Input: part model. Units: mm. Frame: model coordinates. A direction names the side the tool comes from. Round coordinates to 2 decimals unless told otherwise and drop trailing zeros. Write each loop counter-clockwise with the first axis right and the second up, starting at its lowest first coordinate (ties: lowest second). Pieces come first, ordered by that corner, then holes. Notation, with made-up numbers: M 40.5,25 L 78.5,25 A23 cw 78.5,56 Z; hole C 84,8.5 d2. An arc over 180 degrees is marked long. Write each question's results on one line, items separated by ' | '. Start each with the question number.
```python
from build123d import *

# Parameters (mm, degrees)
SKETCH1_W          = 100
SKETCH1_H          = 15
EXTRUDE1_DEPTH     = 15
CUT_EXTRUDE1_DEPTH = 53.737557774
CHAMFER1_SIZE      = 0.5


with BuildPart() as part:
    # Sketch1 → Extrude1 (new body)
    with BuildSketch(Plane(origin=(0, 0, 0), x_dir=(1, 0, 0), z_dir=(0, 1, 0))):
        Rectangle(SKETCH1_W, SKETCH1_H)
    extrude(amount=EXTRUDE1_DEPTH)

    # Sketch4 → Cut-Extrude1 (cut, through all)
    with BuildSketch(Plane(origin=(0, 15, 0), x_dir=(1, 0, 0), z_dir=(0, 1, 0))):
        with BuildLine():
            Line((-42.25, 2.5), (-42.25, -2.5))
            ThreePointArc((-42.25, -2.5), (-40, -4.75), (-37.75, -2.5))
            Line((-37.75, -2.5), (-37.75, 2.5))
            ThreePointArc((-37.75, 2.5), (-40, 4.75), (-42.25, 2.5))
        make_face()
        with BuildLine():
            Line((37.75, 2.5), (37.75, -2.5))
            ThreePointArc((37.75, -2.5), (40, -4.75), (42.25, -2.5))
            Line((42.25, -2.5), (42.25, 2.5))
            ThreePointArc((42.25, 2.5), (40, 4.75), (37.75, 2.5))
        make_face()
    extrude(amount=-CUT_EXTRUDE1_DEPTH, mode=Mode.SUBTRACT)

    # Chamfer1
    chamfer1_edges = [part.edges().sort_by_distance(p)[0] for p in [
        (50, 15, 0),
        (0, 15, -7.5),
        (-50, 15, 0),
        (0, 0, -7.5),
        (50, 0, 0),
        (0, 0, 7.5),
        (-50, 0, 0),
        (0, 15, 7.5),
        (-50, 7.5, -7.5),
        (50, 7.5, -7.5),
        (50, 7.5, 7.5),
        (-50, 7.5, 7.5),
    ]]
    chamfer(chamfer1_edges, length=CHAMFER1_SIZE)


solid = part.part
```
1. Cut plane A-A on z = -1.25. Output: boundary loops of the cut face in (x, y), and give its area (3 significant figures).
2. Draft query along Z for faces 1 (the face through (-37.75, 8, 0)), 2 (the face through (-1, 7, 7.5)), 3 (the face through (37.75, 8, 0)), 4 (the face through (-50, 7, 0)). Return one class per face: +Z half, -Z half, draft (parallel to the pull), parting line (faces both ways), or undercut.
3. Access query for faces 5 (the face through (-1, 0, 0)), 6 (the face through (40.05, 7.6, -4.75)). Directions: +Z, -Z, +X, -X, +Y, -Y. A direction counts if a zero-diameter tool reaches every point of the face in a straight line with its end or side. Return the directions, or none.
4. Cut plane B-B on x = -40. Output: boundary loops of the cut face in (y, z), and give its area (3 significant figures).
5. Line query: L1, parallel to X at y = 8, z = 2.75; L2, parallel to X at y = 8.25, z = -3.75; L3, parallel to Z at x = -38.5, y = 6.25. Output: solid intervals per line, ascending. Write a range as from..to.
6. Cut plane C-C on y = 11.5. Output: boundary loops of the cut face in (x, z), and give its area (3 significant figures).
Answers follow:
1) outline: M -50,0.5 L -49.5,0 L -42.25,0 L -42.25,15 L -49.5,15 L -50,14.5 Z; M -37.75,0 L 37.75,0 L 37.75,15 L -37.75,15 Z; M 42.25,0 L 49.5,0 L 50,0.5 L 50,14.5 L 49.5,15 L 42.25,15 Z | area: 1,360 mm2
2) face 1: undercut | face 2: +Z half | face 3: undercut | face 4: draft
3) face 5: +Z, -Z, +X, -X, -Y | face 6: +Y, -Y
4) outline: M 0,-7 L 0.5,-7.5 L 14.5,-7.5 L 15,-7 L 15,-4.75 L 0,-4.75 Z; M 0,4.75 L 15,4.75 L 15,7 L 14.5,7.5 L 0.5,7.5 L 0,7 Z | area: 82.0 mm2
5) L1: x = -50..-42.24, -37.76..37.76, 42.24..50 | L2: x = -50..-41.87, -38.13..38.13, 41.87..50 | L3: z = -7.5..-4.18, 4.18..7.5
6) outline: M -50,-7 L -49.5,-7.5 L 49.5,-7.5 L 50,-7 L 50,7 L 49.5,7.5 L -49.5,7.5 L -50,7 Z; hole M -42.25,-2.5 A2.25 ccw -37.75,-2.5 L -37.75,2.5 A2.25 ccw -42.25,2.5 Z; hole M 37.75,-2.5 A2.25 ccw 42.25,-2.5 L 42.25,2.5 A2.25 ccw 37.75,2.5 Z | area: 1,420 mm2
